The model under review builds one solid part; all positions refer to its coordinate system, in mm. A direction names the side the tool comes from. Coordinates: 2 decimals unless noted, no trailing zeros. Order: outer loops, then holes, each group sorted by start corner. A loop starts at its lowest first (then second) coordinate and runs counter-clockwise, first axis right, second up. Notation, with made-up numbers: M -36.75,8.5 L -19.75,8.5 A35 ccw -19.75,44.5 Z; hole C 33.25,39.25 d8. An arc over 180 degrees is marked long. Answer in a Markdown table with one row per item.
from build123d import *

# Parameters (mm, degrees)
BOSS_EXTRUDE1_DEPTH = 120
CUT_EXTRUDE1_DEPTH  = 120


with BuildPart() as part:
    # Sketch1 → Boss-Extrude1 (new body)
    with BuildSketch(Plane.XY):
        with BuildLine():
            Line((0, 0), (87, 0))
            ThreePointArc((87, 0), (96.192388155, 3.807611845), (100, 13))
            Line((100, 13), (100, 200))
            Line((100, 200), (92, 200))
            Line((92, 200), (92, 13))
            ThreePointArc((92, 13), (90.535533906, 9.464466094), (87, 8))
            Line((87, 8), (0, 8))
            Line((0, 8), (0, 0))
        make_face()
    extrude(amount=BOSS_EXTRUDE1_DEPTH)

    # Sketch2 → Cut-Extrude1 (cut)
    with BuildSketch(Plane(origin=(0, 8, 0), x_dir=(1, 0, 0), z_dir=(0, 1, 0))):
        with BuildLine():
            Line((12.5, -20.5), (62.5, -20.5))
            ThreePointArc((62.5, -20.5), (67, -25), (62.5, -29.5))
            Line((62.5, -29.5), (12.5, -29.5))
            ThreePointArc((12.5, -29.5), (8, -25), (12.5, -20.5))
        make_face()
        with BuildLine():
            Line((12.5, -99.5), (62.5, -99.5))
            ThreePointArc((62.5, -99.5), (67, -95), (62.5, -90.5))
            Line((62.5, -90.5), (12.5, -90.5))
            ThreePointArc((12.5, -90.5), (8, -95), (12.5, -99.5))
        make_face()
    extrude(amount=-CUT_EXTRUDE1_DEPTH, mode=Mode.SUBTRACT)


solid = part.part
(1) The part is to be moulded in two halves that separate along X. For faces 4 (the flat face through (44, 8, 59)), 5 (the cylindrical face through (8, 4, 95)), 6 (the cylindrical face through (91, 10, 59)), say which applies: +X half, -X half, draft (parallel to the pull), parting line (faces both ways), or undercut.
Report:
| item | result |
|---|---|
| face 4 | draft |
| face 5 | undercut |
| face 6 | -X half |
(2) Take a section at C-C (z = 34.5). Write out the cut boundary in (x, y), then the cut area to 3 significant figures.
Report:
| item | result |
|---|---|
| outline | M 0,0 L 87,0 A13 ccw 100,13 L 100,200 L 92,200 L 92,13 A5 cw 87,8 L 0,8 Z |
| area | 2,310 mm^2 |
(3) Take a section at B-B (x = 52). Write out the cut boundary in (y, z), then the cut area to 3 significant figures.
Report:
| item | result |
|---|---|
| outline | M 0,0 L 8,0 L 8,20.5 L 0,20.5 Z; M 0,29.5 L 8,29.5 L 8,90.5 L 0,90.5 Z; M 0,99.5 L 8,99.5 L 8,120 L 0,120 Z |
| area | 816 mm^2 |
(4) Machinability: for faces 1 (the flat face through (100, 105, 59)), 2 (the cylindrical face through (8, 4, 25)), 3 (the flat face through (92, 108, 59)), which of the approach directions +Z, -Z, +X, -X, +Y, -Y give a long, thin tool a straight path to every point of the face, cutting with its end or side? Answer none if there is none.
Report:
| item | result |
|---|---|
| face 1 | +Z, -Z, +X, +Y, -Y |
| face 2 | +Y, -Y |
| face 3 | +Z, -Z, -X, +Y |
(5) Insertion check: P1, Ø1.5, axis at y = 170.5, z = 52.5, coming from the -X side. The pin has a flat end and moves straight along its axis. Give the tip position at first contact, or say it passes through.
Report:
| item | result |
|---|---|
| P1 | x = 92 |
(6) Take a section at A-A (z = 95). Write out the cut boundary in (x, y).
Report:
| item | result |
|---|---|
| outline | M 0,0 L 8,0 L 8,8 L 0,8 Z; M 67,0 L 87,0 A13 ccw 100,13 L 100,200 L 92,200 L 92,13 A5 cw 87,8 L 67,8 Z |
(7) Take a section at D-D (y = 155). Write out the cut boundary in (x, z), then the cut area to 3 significant figures.
Report:
| item | result |
|---|---|
| outline | M 92,0 L 100,0 L 100,120 L 92,120 Z |
| area | 960 mm^2 |
(8) To check wall thickness, follow line 1 (X direction, y = 20, z = 46.5); line 2 (Y direction, x = 58, z = 51); line 3 (Y direction, x = 92.5, z = 31.5). State the ranges of each line that lie inside material, in increasing order. Write a range as [from, to].
Report:
| item | result |
|---|---|
| line 1 | [92, 100] |
| line 2 | [0, 8] |
| line 3 | [1.22, 200] |
